The model under review builds one solid part; all positions refer to its coordinate system, in mm. Coordinates: 2 decimals unless noted, no trailing zeros. Write each loop counter-clockwise with the first axis right and the second up, starting at its lowest first coordinate (ties: lowest second). Pieces come first, ordered by that corner, then holes. Notation, with made-up numbers: (0, 0) - (46, 0) arc R27 ccw to (46, 38) - close; hole circle Ø1 at (3, -8). An arc over 180 degrees is marked (long way). Put each result on its own line as item: value. Start each with the question number.
Item 1: Mouldability with a two-part tool opening along X and no side actions: class faces 1 (the face through (-31.495, 83.824, 16.381)), 2 (the face through (-37, 170, 0)), 3 (the face through (-25.861, 83.824, -33.727)) as pulls with the +X half, pulls with the -X half, needs draft (parallel to the pull), parting line crosses it, or undercut.
Item 2: For pin 1 (5 mm diameter, centred on y = 79, z = -1, fed in from -X); pin 2 (1 mm diameter, centred on x = -16.5, y = 146.5, fed in from +Z); pin 3 (3 mm diameter, centred on y = 128.5, z = 20.5, fed in from +X), all flat-tipped, find the tip position at first contact; note any pin that passes through.
Item 3: Consider section A-A on x = 0. Give the boundary of the cut face in (y, z).
Item 4: To check wall thickness, follow L1, parallel to X at y = 121, z = 0; L2, parallel to Z at x = -26, y = 39.5; L3, parallel to X at y = 130.5, z = -25. State the ranges of each line that lie inside material, in increasing order. Write a range as [from, to].
Item 5: Consider section C-C on y = 70.5. Give the boundary of the cut face in (x, z), then the cut area to 3 significant figures.
Item 6: Consider section B-B on z = 0. Give the boundary of the cut face in (x, y).
```python
from build123d import *

# Parameters (mm, degrees)
SKETCH1_R           = 42.5
SKETCH1_R_2         = 35.5
BOSS_EXTRUDE1_DEPTH = 170
CHAMFER2_SIZE       = 1


with BuildPart() as part:
    # Sketch1 → Boss-Extrude1 (new body)
    with BuildSketch(Plane(origin=(0, 0, 0), x_dir=(1, 0, 0), z_dir=(0, 1, 0))):
        with Locations(Location((0, 0, 0), (0, 0, 270))):
            Circle(SKETCH1_R)
        with Locations(Location((0, 0, 0), (0, 0, 270))):
            Circle(SKETCH1_R_2, mode=Mode.SUBTRACT)
    extrude(amount=BOSS_EXTRUDE1_DEPTH)

    # Chamfer2
    chamfer2_edges = [part.edges().sort_by_distance(p)[0] for p in [
        (0, 0, -42.5),
        (0, 170, -42.5),
        (0, 0, -35.5),
        (0, 170, -35.5),
    ]]
    chamfer(chamfer2_edges, length=CHAMFER2_SIZE)


solid = part.part
```
Report:
1. face 1: undercut
1. face 2: needs draft
1. face 3: parting line crosses it
2. pin 1: x = -42.5
2. pin 2: z = 39.37
2. pin 3: x = 38.02
3. outline: (0, -41.5) - (1, -42.5) - (169, -42.5) - (170, -41.5) - (170, -36.5) - (169, -35.5) - (1, -35.5) - (0, -36.5) - close; (0, 36.5) - (1, 35.5) - (169, 35.5) - (170, 36.5) - (170, 41.5) - (169, 42.5) - (1, 42.5) - (0, 41.5) - close
4. L1: [-42.5, -35.5], [35.5, 42.5]
4. L2: [-33.62, -24.17], [24.17, 33.62]
4. L3: [-34.37, -25.2], [25.2, 34.37]
5. outline: circle Ø85 at (0, 0); hole circle Ø71 at (0, 0)
5. area: 1,720 mm²
6. outline: (-42.5, 1) - (-41.5, 0) - (-36.5, 0) - (-35.5, 1) - (-35.5, 169) - (-36.5, 170) - (-41.5, 170) - (-42.5, 169) - close; (35.5, 1) - (36.5, 0) - (41.5, 0) - (42.5, 1) - (42.5, 169) - (41.5, 170) - (36.5, 170) - (35.5, 169) - close
